```python
from build123d import *
from OCP.BRepFilletAPI import BRepFilletAPI_MakeChamfer

# Parameters (mm, degrees)
EXTRUDE_1_DEPTH          = 172.5
CUT_EXTRUDE_1_DEPTH      = 196.172359723
CUT_EXTRUDE_1_DEPTH_BACK = 196.172359723
CHAMFER_1_SIZE           = 6
CHAMFER_1_SIZE2          = 6.742931709
CHAMFER_2_SIZE           = 5
CHAMFER_2_SIZE2          = 5.919528387
CHAMFER_2_EDGE_2_SIZE    = 5
CHAMFER_2_EDGE_2_SIZE2   = 5.919528387


with BuildPart() as part:
    # 草图1 → 凸台-拉伸1 (new, symmetric)
    with BuildSketch(Plane.XY):
        Polygon((44, 80), (-44, 80), (-44, 76), (-3, 72), (-3, -72), (-44, -76), (-44, -80), (44, -80), (44, -76), (3, -72), (3, 72), (44, 76), align=None)
    extrude(amount=EXTRUDE_1_DEPTH, both=True)

    # 草图3 → 切除-拉伸1 (cut, two sides: drawn at the far end of the back side and taken through both)
    with BuildSketch(Plane(origin=(0, 0, 0), x_dir=(0, 0, -1), z_dir=(1, 0, 0)).offset(-CUT_EXTRUDE_1_DEPTH_BACK)):
        Polygon((-172.5, 66), (-115.5, 72), (-115.5, 80), (-172.5, 80), align=None)
        Polygon((172.5, 80), (172.5, 66), (131.5, 72), (131.5, 80), align=None)
        Polygon((172.5, -66), (131.5, -72), (131.5, -80), (172.5, -80), align=None)
        Polygon((-172.5, -80), (-172.5, -66), (-115.5, -72), (-115.5, -80), align=None)
    extrude(amount=CUT_EXTRUDE_1_DEPTH + CUT_EXTRUDE_1_DEPTH_BACK, mode=Mode.SUBTRACT)

    # 倒角1: one chamfer whose edges measure the first distance from different faces: ONE call of the kernel's chamfer builder (chamfer() names one face for all edges)
    chamfer_1_edges_1 = [part.edges().sort_by_distance(p)[0] for p in [
        (0, 66, 172.5),
    ]]
    chamfer_1_side_1 = [part.faces().sort_by_distance(p)[0] for p in [
        (0, 69, 144),
    ]]
    chamfer_1_edges_2 = [part.edges().sort_by_distance(p)[0] for p in [
        (0, -66, 172.5),
    ]]
    chamfer_1_side_2 = [part.faces().sort_by_distance(p)[0] for p in [
        (0, -69, 144),
    ]]
    chamfer_1 = BRepFilletAPI_MakeChamfer(part.part.solid().wrapped)
    for e in chamfer_1_edges_1:
        chamfer_1.Add(CHAMFER_1_SIZE, CHAMFER_1_SIZE2, e.wrapped, chamfer_1_side_1[0].wrapped)  # the first distance lies on this face
    for e in chamfer_1_edges_2:
        chamfer_1.Add(CHAMFER_1_SIZE, CHAMFER_1_SIZE2, e.wrapped, chamfer_1_side_2[0].wrapped)  # the first distance lies on this face
    add(Compound.cast(chamfer_1.Shape()), mode=Mode.REPLACE)

    # 倒角2
    chamfer_2_edges = [part.edges().sort_by_distance(p)[0] for p in [
        (0, 66, -172.5),
    ]]
    chamfer_2_side = [part.faces().sort_by_distance(p)[0] for p in [
        (0, 0, -172.5),
    ]]
    chamfer(chamfer_2_edges, length=CHAMFER_2_SIZE, length2=CHAMFER_2_SIZE2, reference=chamfer_2_side[0])

    # 倒角2 edge 2
    chamfer_2_edge_2_edges = [part.edges().sort_by_distance(p)[0] for p in [
        (0, -66, -172.5),
    ]]
    chamfer_2_edge_2_side = [part.faces().sort_by_distance(p)[0] for p in [
        (0, 0, -172.5),
    ]]
    chamfer(chamfer_2_edge_2_edges, length=CHAMFER_2_EDGE_2_SIZE, length2=CHAMFER_2_EDGE_2_SIZE2, reference=chamfer_2_edge_2_side[0])


solid = part.part
```
Geometry check sheet. Reference: the model listing, model coordinates, mm. A direction names the side the tool comes from. Coordinates: 2 decimals unless noted, no trailing zeros. Order: outer loops, then holes, each group sorted by start corner. A loop starts at its lowest first (then second) coordinate and runs counter-clockwise, first axis right, second up. Notation, with made-up numbers: (-20, 51.25) - (-9, 51.25) arc R22 cw to (-9, 83.25) - close; hole circle Ø10 at (65.5, -4.5). An arc over 180 degrees is marked (long way). Answer as a JSON object with one key per item and string values. Group by question number.
Item 1: Sectioned sample at A-A, the plane x = 36. Record the cut outline in (y, z), and give its area (3 significant figures).
Item 2: Sectioned sample at B-B, the plane z = 31.5. Record the cut outline in (x, y), and give its area (3 significant figures).
Item 3: Draft check along Y on faces 4 (the face through (-0.04, -62.89, 169.56)), 5 (the face through (23.79, -74.03, -6.27)), 6 (the face through (-3, 1, 2)), 7 (the face through (-0.042, 69.276, 141.374)). Enter one of: +Y half, -Y half, draft (parallel to the pull), parting line (faces both ways), or undercut.
Item 4: Depth check by flat-ended pin: pin 1 Ø6.5 at (x, y) = (-12.5, 74.5) entering from -Z; pin 2 Ø4 at (x, y) = (8.5, 75.5) entering from +Z; pin 3 Ø1 at (y, z) = (-18, 124) entering from +X. Enter the tip coordinate at first touch or a pass-through.
Item 5: Scan lines: probe 1 along X at (y, z) = (-61.5, -37); probe 2 along Y at (x, z) = (-21.5, -33); probe 3 along Y at (x, z) = (-25, -119.5). Record each from-to range of solid material in increasing order.
Item 6: Tool access check on faces 1 (the face through (-1, 77, -131.5)), 2 (the face through (-1, -77, 115.5)), 3 (the face through (-1, 77, 115.5)). Record the directions out of +Z, -Z, +X, -X, +Y, -Y that give a thin tool (end or side, any length) a straight path to the whole face; none if there is none.
Item 7: Sectioned sample at C-C, the plane x = 13.5. Record the cut outline in (y, z).
Item 8: Sectioned sample at D-D, the plane y = -25.5. Record the cut outline in (x, z).
Resolved:
{
 "1": {"outline": "(-80, -131.5) - (-75.22, -131.5) - (-75.22, 115.5) - (-80, 115.5) - close; (75.22, -131.5) - (80, -131.5) - (80, 115.5) - (75.22, 115.5) - close", "area": "2,360 mm^2"},
 "2": {"outline": "(-44, -80) - (44, -80) - (44, -76) - (3, -72) - (3, 72) - (44, 76) - (44, 80) - (-44, 80) - (-44, 76) - (-3, 72) - (-3, -72) - (-44, -76) - close", "area": "1,940 mm^2"},
 "3": {"face 4": "-Y half", "face 5": "undercut", "face 6": "undercut", "face 7": "+Y half"},
 "4": {"pin 1": "z = -131.5", "pin 2": "z = 115.5", "pin 3": "x = 3"},
 "5": {"probe 1": "-3 to 3", "probe 2": "-80 to -73.8, 73.8 to 80", "probe 3": "-80 to -74.15, 74.15 to 80"},
 "6": {"face 1": "-Z, +X, -X, +Y", "face 2": "+Z, +X, -X, -Y", "face 3": "+Z, +X, -X, +Y"},
 "7": {"outline": "(-80, -131.5) - (-73.02, -131.5) - (-73.02, 115.5) - (-80, 115.5) - close; (73.02, -131.5) - (80, -131.5) - (80, 115.5) - (73.02, 115.5) - close"},
 "8": {"outline": "(-3, -172.5) - (3, -172.5) - (3, 172.5) - (-3, 172.5) - close"}
}
